from build123d import *

# Parameters (mm, degrees)
BASE_PLATE_SKETCH_R = 12.5
BASE_PLATE_DEPTH    = 10
LUG_1_SKETCH_R      = 11
LUG_1_DEPTH         = 10
LUG_2_SKETCH_R      = 11
LUG_2_DEPTH         = 10


with BuildPart() as part:
    # Base Plate Sketch → Base Plate (new body)
    with BuildSketch(Plane(origin=(0, 0, 0), x_dir=(1, 0, 0), z_dir=(0, 1, 0))):
        with BuildLine():
            Line((-19.336184956, -21.171904289), (-25.4662576, -44.368099172))
            Line((-25.4662576, -44.368099172), (0, -71.281889743))
            Line((0, -71.281889743), (27.963619281, -44.368099172))
            Line((27.963619281, -44.368099172), (18.770242682, -19.376964714))
            ThreePointArc((18.770242682, -19.376964714), (-0.941023212, -6.304040126), (-19.336184956, -21.171904289))
        make_face()
        with Locations(Location((0, -26.281889743, 0), (0, 0, 270))):
            Circle(BASE_PLATE_SKETCH_R, mode=Mode.SUBTRACT)
    extrude(amount=BASE_PLATE_DEPTH)

    # Lug 1 Sketch → Lug 1 (add)
    with BuildSketch(Plane(origin=(35.61486713, 0, 37.004099536), x_dir=(0.720502211038311, 0, -0.6934526399754386), z_dir=(0.6934526399754386, 0, 0.720502211038311))):
        with BuildLine():
            Line((-29.430614625, 10), (-29.430614625, 32))
            ThreePointArc((-29.430614625, 32), (-11.430614625, 50), (6.569385375, 32))
            Line((6.569385375, 32), (6.569385375, 10))
            Line((6.569385375, 10), (6.569385375, 0))
            Line((6.569385375, 0), (-29.430614625, 0))
            Line((-29.430614625, 0), (-29.430614625, 10))
        make_face()
        with Locations((-11.430614625, 32)):
            Circle(LUG_1_SKETCH_R, mode=Mode.SUBTRACT)
    extrude(amount=-LUG_1_DEPTH)

    # Lug 2 Sketch → Lug 2 (add)
    with BuildSketch(Plane(origin=(-35.586548141, 0, 33.672559042), x_dir=(0.6873033475884168, 0, 0.7263705035267854), z_dir=(-0.7263705035267854, 0, 0.6873033475884168))):
        with BuildLine():
            Line((31.777062145, 32), (31.777062145, 0))
            Line((31.777062145, 0), (-4.222937855, 0))
            Line((-4.222937855, 0), (-4.222937855, 32))
            ThreePointArc((-4.222937855, 32), (13.777062145, 50), (31.777062145, 32))
        make_face()
        with Locations((13.777062145, 32)):
            Circle(LUG_2_SKETCH_R, mode=Mode.SUBTRACT)
    extrude(amount=-LUG_2_DEPTH)


solid = part.part
Build history of the part. All positions in model axes, mm. A direction names the side the tool comes from. Coordinates: 2 decimals unless noted, no trailing zeros. Write each loop counter-clockwise with the first axis right and the second up, starting at its lowest first coordinate (ties: lowest second). Pieces come first, ordered by that corner, then holes.
(1) Drill centre lines: line 1 (X direction, y = 2.5, z = 31); line 2 (Y direction, x = -1.5, z = 51.5); line 3 (X direction, y = 10.5, z = 32.5). Where is each one in solid material? Low to high.
(2) Cut at D-D on y = 27. List the corners of the cut face in (x, z), and give its area (3 significant figures).
(3) Cut at B-B on x = -3. List the corners of the cut face in (y, z), and give its area (3 significant figures).
(4) Mould opens along Z. For faces 1 (the cylindrical face through (23.675, 49.996, 41.653)), 2 (the cylindrical face through (27.62, 22.24, 37.86)), 3 (the cylindrical face through (-0.59, 4.93, 6.29)), 4 (the cylindrical face through (3.755, 4.93, 38.205)) say: pulls with the +Z half, pulls with the -Z half, needs draft (parallel to the pull), parting line crosses it, or undercut.
(5) 3-axis set-ups, long thin cutter, end or side, ignore diameter. For faces 5 (the flat face through (-20.877, 4.93, 27.001)), 6 (the cylindrical face through (-22.809, 49.996, 40.004)), 7 (the flat face through (-10.2, 21.2, 53.4)), 8 (the flat face through (-18.68, 19.79, 36.99)): which of +Z, -Z, +X, -X, +Y, -Y reach the whole face in a straight line?
(6) Pin check, flat tips, straight feed: pin 1 Ø3 at (x, y) = (-11, 31) entering from +Z; pin 2 Ø1.5 at (y, z) = (16.5, 41) entering from +X; pin 3 Ø2 at (x, z) = (-8, 32) entering from -Y; pin 4 Ø1 at (x, y) = (-12.5, 35.5) entering from -Z. Stop position of each tip, or through.
(7) Cut at C-C on y = 22. List the corners of the cut face in (x, z).
(8) Cut at A-A on y = 14. List the corners of the cut face in (x, z).
Working result:
1. line 1: x = -38.12 to -24.35, -21.93 to -11.58, 11.58 to 23.05, 27.43 to 38.95
1. line 2: y = 0 to 10
1. line 3: x = -36.7 to -22.93, 25.87 to 40.29
2. outline: (-38.49, 30.61) - (-31.23, 23.73) - (-25.59, 29.69) - (-32.85, 36.56) - close; (-19.38, 50.8) - (-12.12, 43.92) - (-6.48, 49.88) - (-13.75, 56.75) - close; (7.48, 50.21) - (13.39, 44.52) - (20.32, 51.73) - (14.41, 57.41) - close; (27.5, 30.93) - (33.41, 25.24) - (40.35, 32.45) - (34.44, 38.14) - close
2. area: 328 mm2
3. outline: (0, 6.51) - (10, 6.51) - (10, 14.15) - (0, 14.15) - close; (0, 38.42) - (10, 38.42) - (10, 68.11) - (0, 68.11) - close
3. area: 373 mm2
4. face 1: parting line crosses it
4. face 2: undercut
4. face 3: pulls with the -Z half
4. face 4: undercut
5. face 5: -Z, +Y, -Y
5. face 6: +Y
5. face 7: +Z, +Y
5. face 8: -Z, +Y
6. pin 1: stops at z = 55.58
6. pin 2: stops at x = 32.24
6. pin 3: passes through
6. pin 4: stops at z = 44.62
7. outline: (-38.49, 30.61) - (-31.23, 23.73) - (-22, 33.48) - (-29.27, 40.35) - close; (-22.97, 47.01) - (-15.7, 40.14) - (-6.48, 49.88) - (-13.75, 56.75) - close; (7.48, 50.21) - (17.14, 40.9) - (24.08, 48.11) - (14.41, 57.41) - close; (23.75, 34.55) - (33.41, 25.24) - (40.35, 32.45) - (30.68, 41.75) - close
8. outline: (-38.49, 30.61) - (-31.23, 23.73) - (-6.48, 49.88) - (-13.75, 56.75) - close; (7.48, 50.21) - (33.41, 25.24) - (40.35, 32.45) - (14.41, 57.41) - close
